Input: part model. Units: mm. Frame: model coordinates. Face numbers are marked on the shaded views. A direction names the side the tool comes from. Coordinates: 2 decimals unless noted, no trailing zeros. Write each loop counter-clockwise with the first axis right and the second up, starting at its lowest first coordinate (ties: lowest second). Pieces come first, ordered by that corner, then holes. Notation, with made-up numbers: (-30, -32.75) - (2, -32.75) arc R24 ccw to (2, 3.25) - close; hole circle Ø6 at (54, 43). An arc over 180 degrees is marked (long way). Use CSV: the item, a comma, the result in double quotes.
```python
from build123d import *

# Parameters (mm, degrees)
SKETCH1_R           = 25
BOSS_EXTRUDE1_DEPTH = 48
SKETCH2_R           = 15
BOSS_EXTRUDE2_DEPTH = 5
BOSS_EXTRUDE3_DEPTH = 15
CHAMFER1_SIZE       = 0.3
SKETCH4_R           = 5.477956266
BOSS_EXTRUDE4_DEPTH = 50
SKETCH5_R           = 1.25
CUT_EXTRUDE1_DEPTH  = 7


with BuildPart() as part:
    # Sketch1 → Boss-Extrude1 (new body)
    with BuildSketch(Plane.XY):
        Circle(SKETCH1_R)
    extrude(amount=BOSS_EXTRUDE1_DEPTH)

    # Sketch2 → Boss-Extrude2 (add)
    with BuildSketch(Plane.XY.offset(48)):
        Circle(SKETCH2_R)
    extrude(amount=BOSS_EXTRUDE2_DEPTH)

    # Sketch3 → Boss-Extrude3 (add)
    with BuildSketch(Plane.XY.offset(53)):
        with BuildLine():
            Line((-2.645751311, 3), (2.645751311, 3))
            ThreePointArc((2.645751311, 3), (0, -4), (-2.645751311, 3))
        make_face()
    extrude(amount=BOSS_EXTRUDE3_DEPTH)

    # Chamfer1
    chamfer1_edges = [part.edges().sort_by_distance(p)[0] for p in [
        (0, -4, 68),
        (0, 3, 68),
    ]]
    chamfer(chamfer1_edges, length=CHAMFER1_SIZE)

    # Sketch4 → Boss-Extrude4 (add)
    with BuildSketch(Plane(origin=(0, 0, 0), x_dir=(1, 0, 0), z_dir=(0, 1, 0))):
        with Locations(Location((0, -7.083492504, 0), (0, 0, 90))):
            Circle(SKETCH4_R)
    extrude(amount=BOSS_EXTRUDE4_DEPTH)

    # Sketch5 → Cut-Extrude1 (cut)
    with BuildSketch(Plane.XY.offset(48)):
        with Locations((0, 20)):
            Circle(SKETCH5_R)
        with Locations((17.320508076, 10)):
            Circle(SKETCH5_R)
        with Locations((17.320508076, -10)):
            Circle(SKETCH5_R)
        with Locations((0, -20)):
            Circle(SKETCH5_R)
        with Locations((-17.320508076, -10)):
            Circle(SKETCH5_R)
        with Locations((-17.320508076, 10)):
            Circle(SKETCH5_R)
    extrude(amount=-CUT_EXTRUDE1_DEPTH, mode=Mode.SUBTRACT)


solid = part.part
```
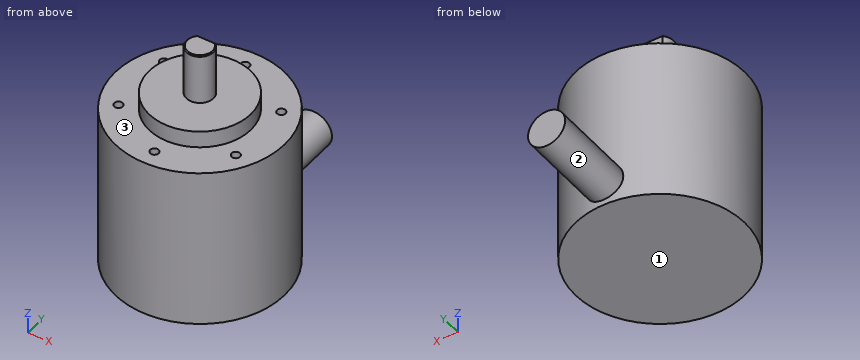
(1) Cut plane B-B on x = 0. Return loops of the section in (y, z).
Check values:
outline,"(-25, 0) - (25, 0) - (25, 1.61) - (50, 1.61) - (50, 12.56) - (25, 12.56) - (25, 48) - (21.25, 48) - (21.25, 41) - (18.75, 41) - (18.75, 48) - (15, 48) - (15, 53) - (3, 53) - (3, 67.7) - (2.7, 68) - (-3.7, 68) - (-4, 67.7) - (-4, 53) - (-15, 53) - (-15, 48) - (-18.75, 48) - (-18.75, 41) - (-21.25, 41) - (-21.25, 48) - (-25, 48) - close"
(2) Reachability of the marked faces 1, 2 and 3 from +Z, -Z, +X, -X, +Y, -Y: full face, straight path, thin tool, end or side. Return the list, or none.
Check values:
face 1,"-Z, +X, -X, +Y, -Y"
face 2,"+Y"
face 3,"+Z"
(3) Ray query, probe 1 along Y at (x, z) = (0, 43.25); probe 2 along Z at (x, y) = (-11, 7); probe 3 along Z at (x, y) = (-10.5, -14). Return the intervals inside material, ascending. Write a range as from..to.
Check values:
probe 1,"-25..-21.25, -18.75..18.75, 21.25..25"
probe 2,"0..53"
probe 3,"0..48"
(4) Cut plane A-A on y = -20. Return loops of the section in (x, z).
Check values:
outline,"(-15, 0) - (15, 0) - (15, 48) - (1.25, 48) - (1.25, 41) - (-1.25, 41) - (-1.25, 48) - (-15, 48) - close"
(5) Pin query (flat end, axial travel): pin 1 Ø0.8 at (x, y) = (-17.5, 10) entering from +Z; pin 2 Ø4 at (x, z) = (-15.5, 33.5) entering from +Y; pin 3 Ø1.2 at (x, y) = (-18, -9.5) entering from +Z; pin 4 Ø15 at (x, y) = (-4.5, 4.5) entering from +Z. Return the tip coordinate at first contact, or that it passes through.
Check values:
pin 1,"z = 41"
pin 2,"y = 21.04"
pin 3,"z = 48"
pin 4,"z = 68"
(6) Cut plane D-D on y = -10. Return loops of the section in (x, z), and give its area (3 significant figures).
Check values:
outline,"(-22.91, 0) - (22.91, 0) - (22.91, 48) - (18.57, 48) - (18.57, 41) - (16.07, 41) - (16.07, 48) - (11.18, 48) - (11.18, 53) - (-11.18, 53) - (-11.18, 48) - (-16.07, 48) - (-16.07, 41) - (-18.57, 41) - (-18.57, 48) - (-22.91, 48) - close"
area,"2,280 mm^2"
(7) Cut plane C-C on z = 13.5. Return loops of the section in (x, y), and give its area (3 significant figures).
Check values:
outline,"circle Ø50 at (0, 0)"
area,"1,960 mm^2"
